Job drawing, mm, ordinate dimensions from the low corner. One solid piece. Give positions to 0.01 mm unless a question says otherwise; leave off trailing zeros. Write each loop counter-clockwise with the first axis right and the second up, starting at its lowest first coordinate (ties: lowest second). Pieces come first, ordered by that corner, then holes. Notation, with made-up numbers: (55.5, 8.25) -> (112.5, 8.25) arc R22 cw to (112.5, 39.25) -> close; hole circle Ø1 at (59, 89). An arc over 180 degrees is marked (long way). Put each result on its own line as item: value. Start each with the question number.
Item 1: Slice it at B-B, the plane y = 2.4. List the corners of the cut face in (x, z).
Item 2: Drill centre lines: line 1 along X through (y, z) = (2.9, 25); line 2 along X through (y, z) = (4.05, 25); line 3 along Z through (x, y) = (7.5, 3.2). Where is each one in solid material? Low to high.
Item 3: Two-plate mould, pull along Z, no slides. Class the marked faces 1 and 2: pulls with the +Z half, pulls with the -Z half, needs draft (parallel to the pull), parting line crosses it, or undercut.
Item 4: Flat gauge pins, fed straight in: pin 1 Ø2 at (x, y) = (34, 1) entering from +Z; pin 2 Ø3 at (x, y) = (10.5, 1.5) entering from +Z. Where does each tip first touch, or does it go through?
Item 5: Slice it at A-A, the plane z = 25. List the corners of the cut face in (x, y), plus the area to 3 significant figures.
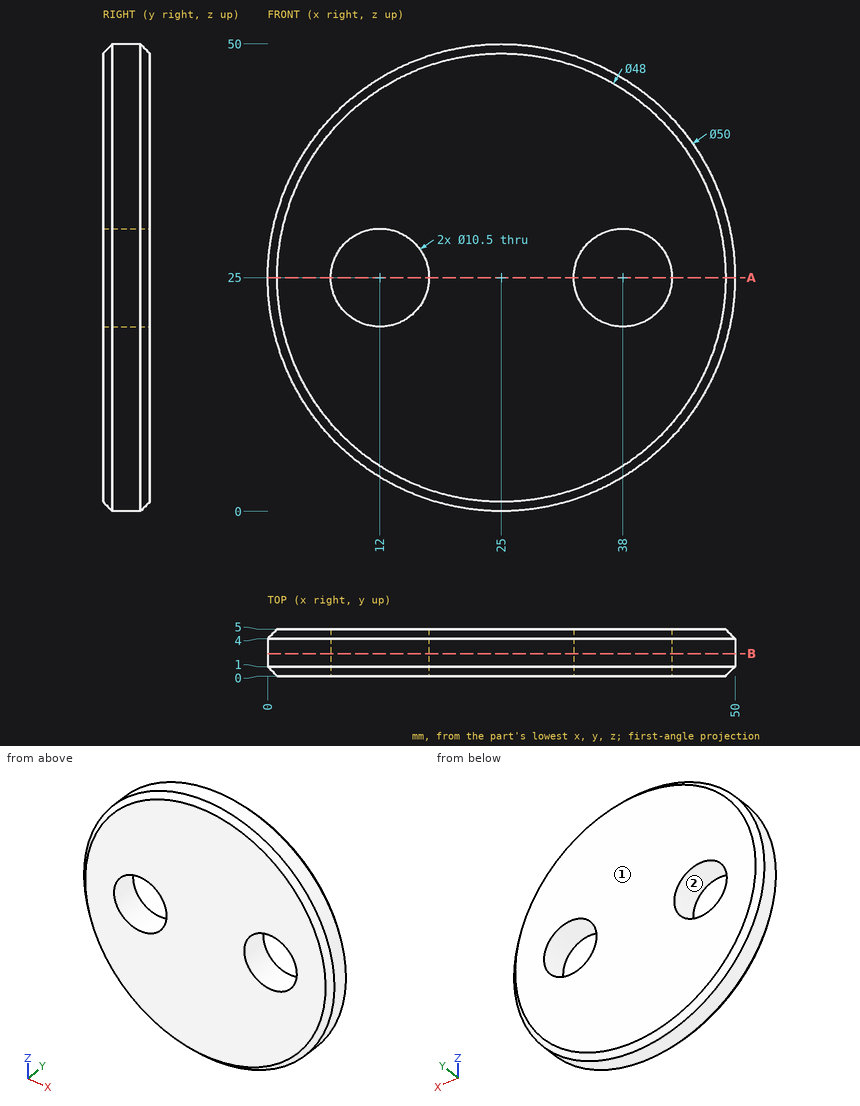
Values follow:
1. outline: circle Ø50 at (25, 25); hole circle Ø10.5 at (12, 25); hole circle Ø10.5 at (38, 25)
2. line 1: 0 to 6.75, 17.25 to 32.75, 43.25 to 50
2. line 2: 0.05 to 6.75, 17.25 to 32.75, 43.25 to 49.95
2. line 3: 7.15 to 22.3, 27.7 to 42.85
3. face 1: needs draft
3. face 2: undercut
4. pin 1: z = 48.69
4. pin 2: z = 46.35
5. outline: (0, 1) -> (1, 0) -> (6.75, 0) -> (6.75, 5) -> (1, 5) -> (0, 4) -> close; (17.25, 0) -> (32.75, 0) -> (32.75, 5) -> (17.25, 5) -> close; (43.25, 0) -> (49, 0) -> (50, 1) -> (50, 4) -> (49, 5) -> (43.25, 5) -> close
5. area: 143 mm2
